```python
from build123d import *

# Parameters (mm, degrees)
BOSS_EXTRUDE1_DEPTH = 5
SKETCH2_R           = 2.5
CUT_EXTRUDE1_DEPTH  = 5
SKETCH3_OUTSIDE_W   = 21.092
SKETCH3_OUTSIDE_H   = 19.7
SKETCH3_OUTSIDE_R   = 4.5
CUT_EXTRUDE2_DEPTH  = 5
CUT_EXTRUDE2_DRAFT  = -30
SKETCH4_OUTSIDE_W   = 21.092
SKETCH4_OUTSIDE_H   = 19.7
SKETCH4_OUTSIDE_R   = 4.5
CUT_EXTRUDE3_DEPTH  = 5
CUT_EXTRUDE3_DRAFT  = -30
CHAMFER1_SIZE       = 0.5
CHAMFER2_SIZE       = 0.5


with BuildPart() as part:
    # Sketch1 → Boss-Extrude1 (new body)
    with BuildSketch(Plane(origin=(0, 0, 0), x_dir=(1, 0, 0), z_dir=(0, 1, 0))):
        Polygon((2.598076211, 4.5), (-2.598076211, 4.5), (-5.196152423, 0), (-2.598076211, -4.5), (2.598076211, -4.5), (5.196152423, 0), align=None)
    extrude(amount=BOSS_EXTRUDE1_DEPTH)

    # Sketch2 → Cut-Extrude1 (cut)
    with BuildSketch(Plane(origin=(0, 5, 0), x_dir=(1, 0, 0), z_dir=(0, 1, 0))):
        with Locations(Location((0, 0, 0), (0, 0, 270))):
            Circle(SKETCH2_R)
    extrude(amount=-CUT_EXTRUDE1_DEPTH, mode=Mode.SUBTRACT)


with BuildPart() as cut_extrude2_tool:
    # Sketch3 outside → Cut-Extrude2 (with draft: the straight prism first)
    with BuildSketch(Plane(origin=(0, 5, 0), x_dir=(1, 0, 0), z_dir=(0, 1, 0))):
        Rectangle(SKETCH3_OUTSIDE_W, SKETCH3_OUTSIDE_H)
        Circle(SKETCH3_OUTSIDE_R, mode=Mode.SUBTRACT)
    extrude(amount=-CUT_EXTRUDE2_DEPTH)
    # Cut-Extrude2: the draft: its side faces are tilted about the plane it starts from
    cut_extrude2_sides = [cut_extrude2_tool.faces().sort_by_distance(p)[0] for p in [
        (0, 2.5, 9.85),
        (10.546, 2.5, 0),
        (0, 2.5, -9.85),
        (-10.546, 2.5, 0),
        (-4.5, 2.5, 0),
    ]]
    draft(cut_extrude2_sides, Plane(origin=(0, 5, 0), x_dir=(1, 0, 0), z_dir=(0, 1, 0)), CUT_EXTRUDE2_DRAFT)


with BuildPart() as part_1:
    add(part.part)

    # Cut-Extrude2: cut by cut_extrude2_tool
    add(cut_extrude2_tool.part, mode=Mode.SUBTRACT)


with BuildPart() as cut_extrude3_tool:
    # Sketch4 outside → Cut-Extrude3 (with draft: the straight prism first)
    with BuildSketch(Plane.XZ):
        Rectangle(SKETCH4_OUTSIDE_W, SKETCH4_OUTSIDE_H)
        Circle(SKETCH4_OUTSIDE_R, mode=Mode.SUBTRACT)
    extrude(amount=-CUT_EXTRUDE3_DEPTH)
    # Cut-Extrude3: the draft: its side faces are tilted about the plane it starts from
    cut_extrude3_sides = [cut_extrude3_tool.faces().sort_by_distance(p)[0] for p in [
        (0, 2.5, -9.85),
        (10.546, 2.5, 0),
        (0, 2.5, 9.85),
        (-10.546, 2.5, 0),
        (-4.5, 2.5, 0),
    ]]
    draft(cut_extrude3_sides, Plane.XZ, CUT_EXTRUDE3_DRAFT)


with BuildPart() as part_2:
    add(part_1.part)

    # Cut-Extrude3: cut by cut_extrude3_tool
    add(cut_extrude3_tool.part, mode=Mode.SUBTRACT)

    # Chamfer1
    chamfer1_edges = [part_2.edges().sort_by_distance(p)[0] for p in [
        (0, 5, -2.5),
    ]]
    chamfer(chamfer1_edges, length=CHAMFER1_SIZE)

    # Chamfer2
    chamfer2_edges = [part_2.edges().sort_by_distance(p)[0] for p in [
        (0, 0, -2.5),
    ]]
    chamfer(chamfer2_edges, length=CHAMFER2_SIZE)


solid = part_2.part
```
CAD build for the part. Positions are in the model's coordinates, mm. Round coordinates to 2 decimals unless told otherwise and drop trailing zeros. Write each loop counter-clockwise with the first axis right and the second up, starting at its lowest first coordinate (ties: lowest second). Pieces come first, ordered by that corner, then holes.
Item 1: Drop flat-ended pins along their axis: pin 1 Ø1.5 at (y, z) = (1, -1) entering from +X; pin 2 Ø2 at (x, y) = (-4, 3) entering from +Z. Give the stop position or say it passes through.
Filled in:
pin 1: stops at x = 5.05
pin 2: stops at z = 3.8
Item 2: Drill centre lines: L1, parallel to X at y = 4.15, z = -1; L2, parallel to Z at x = 0.75, y = 3.85; L3, parallel to X at y = 2.25, z = 1.75. Where is each one in solid material? Low to high.
Filled in:
L1: x = -4.62 to -2.29, 2.29 to 4.62
L2: z = -4.5 to -2.38, 2.38 to 4.5
L3: x = -4.19 to -1.79, 1.79 to 4.19
Item 3: Band-saw the part on A-A on y = 3.5. Write the cut outline in (x, z).
Filled in:
outline: (-5.2, 0) - (-2.6, -4.5) - (2.6, -4.5) - (5.2, 0) - (2.6, 4.5) - (-2.6, 4.5) - close; hole circle Ø5 at (0, 0)
Item 4: Mould opens along Z. For faces 1 (the cylindrical face through (-2.44, 2.53, -0.54)), 2 (the conical face through (2.34, 4.71, -4.04)), 3 (the conical face through (4.666, 0.287, -0.011)) say: released by +Z, released by -Z, zero draft, split by the parting line, or undercut.
Filled in:
face 1: undercut
face 2: released by -Z
face 3: split by the parting line
